from build123d import *

# Parameters (mm, degrees)
BOSS_EXTRUDE1_DEPTH = 10
SKETCH3_R           = 7
CUT_EXTRUDE1_DEPTH  = 10


with BuildPart() as part:
    # Sketch1 → Boss-Extrude1 (new body)
    with BuildSketch(Plane.XY):
        Polygon((12.124355653, 0), (6.062177826, 10.5), (-6.062177826, 10.5), (-12.124355653, 0), (-6.062177826, -10.5), (6.062177826, -10.5), align=None)
    extrude(amount=BOSS_EXTRUDE1_DEPTH)

    # Sketch2 → Cut-Revolve1 (revolve, cut)
    with BuildSketch(Plane(origin=(0, 0, 0), x_dir=(1, 0, 0), z_dir=(0, 1, 0))):
        with BuildLine():
            Line((-12.124355653, 0), (-12.124355653, -1))
            ThreePointArc((-12.124355653, -1), (-10.705494483, -0.25658351), (-9.124355653, 0))
            Line((-9.124355653, 0), (-12.124355653, 0))
        make_face()
        with BuildLine():
            Line((-12.124355653, -10), (-12.124355653, -9))
            ThreePointArc((-12.124355653, -9), (-10.705494483, -9.74341649), (-9.124355653, -10))
            Line((-9.124355653, -10), (-12.124355653, -10))
        make_face()
    revolve(axis=Axis((0, 0, 0), (0, 0, 1)), mode=Mode.SUBTRACT)

    # Sketch3 → Cut-Extrude1 (cut)
    with BuildSketch(Plane(origin=(0, 0, 0), x_dir=(-1, 0, 0), z_dir=(0, 0, -1))):
        Circle(SKETCH3_R)
    extrude(amount=-CUT_EXTRUDE1_DEPTH, mode=Mode.SUBTRACT)


solid = part.part
CAD build for the part. Positions are in the model's coordinates, mm. Round coordinates to 2 decimals unless told otherwise and drop trailing zeros. Loops run counter-clockwise (first coordinate to the right, second up) from the corner with the lowest first, then second, coordinate; pieces in that order, holes last. Notation, with made-up numbers: (21, 53) - (62, 53) arc R16 ccw to (62, 58) - close; hole circle Ø1 at (36.5, -21.75). An arc over 180 degrees is marked (long way). Put each result on its own line as item: value.
1. Slice it at B-B on z = 6.5. List the corners of the cut face in (x, y), and give its area (3 significant figures).
Geometry check:
outline: (-12.12, 0) - (-6.06, -10.5) - (6.06, -10.5) - (12.12, 0) - (6.06, 10.5) - (-6.06, 10.5) - close; hole circle Ø14 at (0, 0)
area: 228 mm²
2. Wall check: line 1 (Y direction, x = 0, z = 6); line 2 (X direction, y = -2.75, z = 2.5); line 3 (X direction, y = 5.75, z = 7). Give the ranges that are in metal, low to high.
Geometry check:
line 1: -10.5 to -7, 7 to 10.5
line 2: -10.54 to -6.44, 6.44 to 10.54
line 3: -8.8 to -3.99, 3.99 to 8.8
3. Two-plate mould, pull along X, no slides. Class faces 1 (the cylindrical face through (-6.466, -2.681, 4.93)), 2 (the flat face through (0, 10.5, 5)), 3 (the flat face through (-9.051, 5.324, 4.933)), 4 (the flat face through (9.136, 5.177, 4.933)): released by +X, released by -X, zero draft, split by the parting line, or undercut.
Geometry check:
face 1: undercut
face 2: zero draft
face 3: released by -X
face 4: released by +X
4. Slice it at A-A on x = 0. List the corners of the cut face in (y, z), and give its area (3 significant figures).
Geometry check:
outline: (-10.5, 0.19) arc R5 ccw to (-9.12, 0) - (-7, 0) - (-7, 10) - (-9.12, 10) arc R5 ccw to (-10.5, 9.81) - close; (7, 0) - (9.12, 0) arc R5 ccw to (10.5, 0.19) - (10.5, 9.81) arc R5 ccw to (9.12, 10) - (7, 10) - close
area: 69.6 mm²
5. Pin check, flat tips, straight feed: P1, Ø1, axis at y = -6.5, z = 4, coming from the -X side; P2, Ø1, axis at x = -9.5, z = 2, coming from the +Y side; P3, Ø6, axis at x = 2, y = 5.5, coming from the +Z side; P4, Ø1, axis at x = 8, z = 7, coming from the -Y side. Stop position of each tip, or through.
Geometry check:
P1: x = -8.66
P2: y = 5.41
P3: z = 10
P4: y = -8.01
